Input: dimensioned drawing with shaded views. Units: mm. Origin: part minimum x, y, z. A direction names the side the tool comes from. Round coordinates to 2 decimals unless told otherwise and drop trailing zeros. Write each loop counter-clockwise with the first axis right and the second up, starting at its lowest first coordinate (ties: lowest second). Pieces come first, ordered by that corner, then holes. Notation, with made-up numbers: M -8.5,25.25 L 32.5,25.25 A7 ccw 32.5,37.25 Z; hole C 59,53.5 d7. An arc over 180 degrees is marked long. Put each result on its own line as item: value. Start each with the question number.
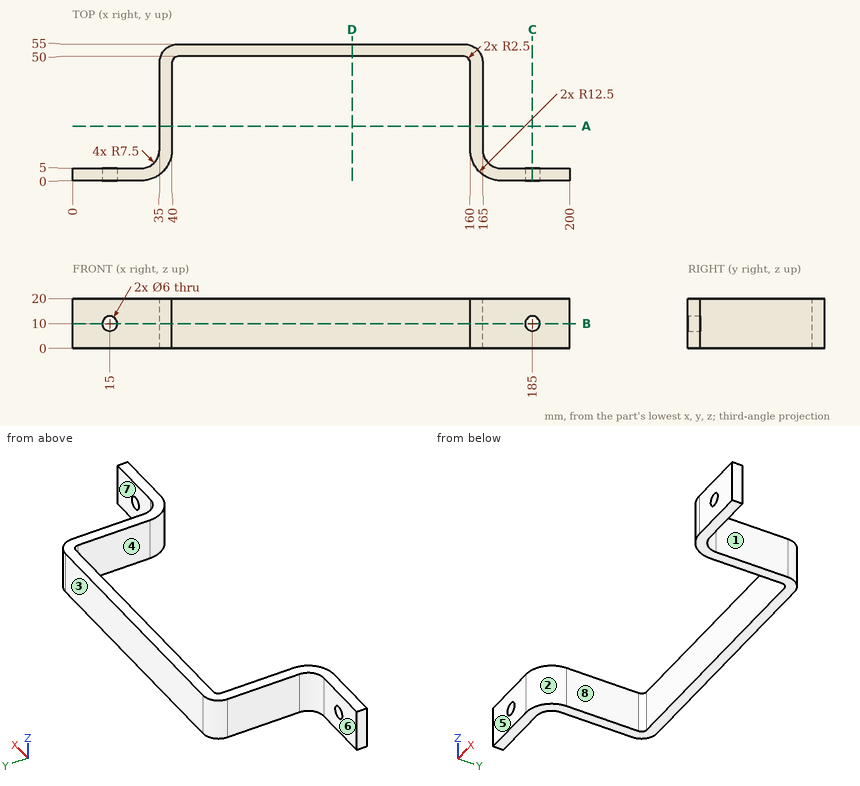
1) Access query for the marked faces 5, 6, 7 and 8. Directions: +Z, -Z, +X, -X, +Y, -Y. A direction counts if a zero-diameter tool reaches every point of the face in a straight line with its end or side. Return the directions, or none.
2) Section B-B, the plane z = 10. Output: boundary loops of the cut face in (x, y), and give its area (3 significant figures).
3) Ray query, probe 1 along X at (y, z) = (47.5, 5.75); probe 2 along X at (y, z) = (3.05, 10); probe 3 along Y at (x, z) = (123, 16.75). Return the intervals inside material, ascending.
4) First-contact query: pin 1 (7 mm diameter, centred on x = 15, z = 10, fed in from -Y); pin 2 (12 mm diameter, centred on y = 35.5, z = 3.5, fed in from +X); pin 3 (8 mm diameter, centred on y = 16, z = 12, fed in from -X); pin 4 (8 mm diameter, centred on x = 73, z = 14.5, fed in from -Y). Flat tips, straight axial feed; report the tip coordinate or a pass-through.
5) Section D-D, the plane x = 112.5. Output: boundary loops of the cut face in (y, z).
6) Section C-C, the plane x = 185. Output: boundary loops of the cut face in (y, z).
7) Draft query along X for the marked faces 1, 2, 3 and 4. Return one class per face: +X half, -X half, draft (parallel to the pull), parting line (faces both ways), or undercut.
8) Section A-A, the plane y = 22. Output: boundary loops of the cut face in (x, z), and give its area (3 significant figures).
Solved:
1. face 5: +Z, -Z, +X, -X, -Y
1. face 6: +Z, -Z, -X, +Y
1. face 7: +Z, -Z, +X, +Y
1. face 8: +Z, -Z, -Y
2. outline: M 0,0 L 12,0 L 12,5 L 0,5 Z; M 18,0 L 27.5,0 A12.5 ccw 40,12.5 L 40,47.5 A2.5 cw 42.5,50 L 157.5,50 A2.5 cw 160,47.5 L 160,12.5 A12.5 ccw 172.5,0 L 182,0 L 182,5 L 172.5,5 A7.5 cw 165,12.5 L 165,47.5 A7.5 ccw 157.5,55 L 42.5,55 A7.5 ccw 35,47.5 L 35,12.5 A7.5 cw 27.5,5 L 18,5 Z; M 188,0 L 200,0 L 200,5 L 188,5 Z
2. area: 1,380 mm2
3. probe 1: x = 35 to 40, 160 to 165
3. probe 2: x = 0 to 12, 18 to 35.68, 164.32 to 182, 188 to 200
3. probe 3: y = 50 to 55
4. pin 1: stops at y = 0
4. pin 2: stops at x = 165
4. pin 3: stops at x = 34.98
4. pin 4: stops at y = 50
5. outline: M 50,0 L 55,0 L 55,20 L 50,20 Z
6. outline: M 0,0 L 5,0 L 5,7 L 0,7 Z; M 0,13 L 5,13 L 5,20 L 0,20 Z
7. face 1: +X half
7. face 2: undercut
7. face 3: draft
7. face 4: undercut
8. outline: M 35,0 L 40,0 L 40,20 L 35,20 Z; M 160,0 L 165,0 L 165,20 L 160,20 Z
8. area: 200 mm2
